Build history of the part. All positions in model axes, mm. A direction names the side the tool comes from. Give positions to 0.01 mm unless a question says otherwise; leave off trailing zeros. Loops run counter-clockwise (first coordinate to the right, second up) from the corner with the lowest first, then second, coordinate; pieces in that order, holes last. Notation, with made-up numbers: (1, -21.5) -> (43, -21.5) arc R23 cw to (43, -10.5) -> close; hole circle Ø3 at (61.5, 4). An arc over 180 degrees is marked (long way). Answer as a JSON object with one key per item and string values. Group by question number.
from build123d import *

# Parameters (mm, degrees)
OVAL_PLATE_DEPTH           = 8
PIN_BOSS_SKETCH_R          = 8
PIN_BOSS_DEPTH             = 6
REAR_START                 = 12
REAR_BOSS_SKETCH_R         = 8
REAR_BOSS_DEPTH            = 12
TUBE_NECK_SKETCH_R         = 13
TUBE_NECK_26_DEPTH         = 16
TUBE_BOSS_SKETCH_R         = 16
TUBE_BOSS_32_DEPTH         = 16
TUBE_START                 = -15
TUBE_BORE_SKETCH_R         = 13
TUBE_BORE_26_DEPTH         = 15
TUBE_NECK_ROOT_FILLET_R3_R = 3
PIN_BOSS_CHAMFER_2MM_SIZE  = 2
PIN_HOLE_SKETCH_R          = 4
PIN_THROUGH_HOLE_DEPTH     = 50


with BuildPart() as part:
    # Oval Plate Sketch → Oval Plate (new body)
    with BuildSketch(Plane.XY):
        with BuildLine():
            Line((-40, 11.313708499), (-8, 22.627416998))
            ThreePointArc((-8, 22.627416998), (24, 0), (-8, -22.627416998))
            Line((-8, -22.627416998), (-40, -11.313708499))
            ThreePointArc((-40, -11.313708499), (-48, 0), (-40, 11.313708499))
        make_face()
    extrude(amount=OVAL_PLATE_DEPTH)

    # Pin Boss Sketch → Pin Boss (add)
    with BuildSketch(Plane.XY.offset(8)):
        with Locations((-36, 0)):
            Circle(PIN_BOSS_SKETCH_R)
    extrude(amount=PIN_BOSS_DEPTH)

    # Rear Boss Sketch → Rear Boss (add)
    with BuildSketch(Plane(origin=(0, 0, 0), x_dir=(-1, 0, 0), z_dir=(0, 0, -1)).offset(REAR_START)):
        with Locations(Location((36, 0, 0), (0, 0, 180))):
            Circle(REAR_BOSS_SKETCH_R)
    extrude(amount=-REAR_BOSS_DEPTH)

    # Tube Neck Sketch → Tube Neck Ø26 (add)
    with BuildSketch(Plane.XY.offset(8)):
        Circle(TUBE_NECK_SKETCH_R)
    extrude(amount=TUBE_NECK_26_DEPTH)

    # Tube Boss Sketch → Tube Boss Ø32 (add)
    with BuildSketch(Plane.XY.offset(24)):
        Circle(TUBE_BOSS_SKETCH_R)
    extrude(amount=TUBE_BOSS_32_DEPTH)

    # Tube Bore Sketch → Tube Bore Ø26 (cut)
    with BuildSketch(Plane.XY.offset(40).offset(TUBE_START)):
        Circle(TUBE_BORE_SKETCH_R)
    extrude(amount=TUBE_BORE_26_DEPTH, mode=Mode.SUBTRACT)

    # Tube Neck Root Fillet R3
    tube_neck_root_fillet_r3_edges = [part.edges().sort_by_distance(p)[0] for p in [
        (-13, 0, 8),
    ]]
    fillet(tube_neck_root_fillet_r3_edges, radius=TUBE_NECK_ROOT_FILLET_R3_R)

    # Pin Boss Chamfer 2mm
    pin_boss_chamfer_2mm_edges = [part.edges().sort_by_distance(p)[0] for p in [
        (-44, 0, 8),
    ]]
    chamfer(pin_boss_chamfer_2mm_edges, length=PIN_BOSS_CHAMFER_2MM_SIZE)

    # Pin Hole Sketch → Pin Through Hole (cut)
    with BuildSketch(Plane.XY.offset(14)):
        with Locations((-36, 0)):
            Circle(PIN_HOLE_SKETCH_R)
    extrude(amount=-PIN_THROUGH_HOLE_DEPTH, mode=Mode.SUBTRACT)


solid = part.part
(1) Probe line 1 along Y through (x, z) = (-36, -5.5); line 2 along Y through (x, z) = (0, 30.5); line 3 along X through (y, z) = (3, 3). List the from-to ranges inside material, lowest first. Write a range as [from, to].
(2) Pin check, flat tips, straight feed: pin 1 (1 mm diameter, centred on x = 4, y = 12, fed in from +Z); pin 2 (2 mm diameter, centred on y = -3.5, z = -5.5, fed in from -X); pin 3 (5 mm diameter, centred on x = -17, y = 10, fed in from +Z); pin 4 (8 mm diameter, centred on x = -0.5, y = 1, fed in from +Z). Stop position of each tip, or through.
(3) Pull direction Z, two halves, no side cores. Call faces 6 (the flat face through (-1.3, 13.1, 24)), 7 (the cylindrical face through (-48, 0, 4)), 8 (the flat face through (-3, 0, 0)): pulls with the +Z half, pulls with the -Z half, needs draft (parallel to the pull), parting line crosses it, or undercut.
(4) Saw through at C-C on z = -6.5. List the corners of the cut face in (x, y).
(5) 3-axis set-ups, long thin cutter, end or side, ignore diameter. For faces 1 (the cylindrical face through (-42.349, 4.868, -6.084)), 2 (the flat face through (-40, -2, 14)), 3 (the flat face through (-1.3, 13.1, 40)), 4 (the cylindrical face through (-10.316, -7.91, 32.395)), 5 (the cylindrical face through (-10.316, -7.91, 17.409)): which of +Z, -Z, +X, -X, +Y, -Y reach the whole face in a straight line?
(6) Saw through at D-D on x = 0. List the corners of the cut face in (y, z).
(7) Saw through at B-B on x = -36. List the corners of the cut face in (y, z), plus the area to 3 significant figures.
Calculated:
{
 "1": {"line 1": "y = [-8, -4], [4, 8]", "line 2": "y = [-16, -13], [13, 16]", "line 3": "x = [-47.62, -38.65], [-33.35, 23.81]"},
 "2": {"pin 1": "stops at z = 40", "pin 2": "stops at x = -43.6", "pin 3": "stops at z = 8", "pin 4": "stops at z = 25"},
 "3": {"face 6": "undercut", "face 7": "needs draft", "face 8": "pulls with the -Z half"},
 "4": {"outline": "circle Ø16 at (-36, 0); hole circle Ø8 at (-36, 0)"},
 "5": {"face 1": "-Z", "face 2": "+Z, -X, +Y, -Y", "face 3": "+Z, +X, -X, +Y, -Y", "face 4": "+Z", "face 5": "none"},
 "6": {"outline": "(-24, 0) -> (24, 0) -> (24, 8) -> (16, 8) arc R3 cw to (13, 11) -> (13, 24) -> (16, 24) -> (16, 40) -> (13, 40) -> (13, 25) -> (-13, 25) -> (-13, 40) -> (-16, 40) -> (-16, 24) -> (-13, 24) -> (-13, 11) arc R3 cw to (-16, 8) -> (-24, 8) -> close"},
 "7": {"outline": "(-12.73, 0) -> (-8, 0) -> (-8, -12) -> (-4, -12) -> (-4, 14) -> (-8, 14) -> (-8, 10) -> (-10, 8) -> (-12.73, 8) -> close; (4, -12) -> (8, -12) -> (8, 0) -> (12.73, 0) -> (12.73, 8) -> (10, 8) -> (8, 10) -> (8, 14) -> (4, 14) -> close", "area": "288 mm^2"}
}
